Part model, mm, in its own coordinate system. A direction names the side the tool comes from. Round coordinates to 2 decimals unless told otherwise and drop trailing zeros. Write each loop counter-clockwise with the first axis right and the second up, starting at its lowest first coordinate (ties: lowest second). Pieces come first, ordered by that corner, then holes.
from build123d import *

# Parameters (mm, degrees)
SKETCH_2_R          = 2.1
CUT_EXTRUDE_1_DEPTH = 48.333920184
SKETCH_3_R          = 2.1
CUT_EXTRUDE_2_DEPTH = 53.389073288
EXTRUDE_1_DEPTH     = 4
FILLET_1_R          = 5


with BuildPart() as part:
    # 草图1 → 旋转1 (revolve)
    with BuildSketch(Plane(origin=(0, 0, 0), x_dir=(1, 0, 0), z_dir=(0, 1, 0)), mode=Mode.PRIVATE) as revolve_1_sk:
        Polygon((0, 21.25), (0, 23.75), (12, 23.75), (12, 31.5), (16, 31.5), (16, 23.75), (29.45, 23.75), (29.45, 13.01), (25.45, 13.01), (25.45, 21.25), align=None)
    revolve(revolve_1_sk.sketch.rotate(Axis((-873.269597079, 0, 0), (1, 0, 0)), 180), axis=Axis((-873.269597079, 0, 0), (1, 0, 0)))

    # 草图2 → 切除-拉伸1 (cut, through all)
    with BuildSketch(Plane(origin=(16, 0, 0), x_dir=(0, 0, -1), z_dir=(1, 0, 0))):
        with Locations((0, 27.75)):
            Circle(SKETCH_2_R)
        with Locations((-24.032204955, 13.875)):
            Circle(SKETCH_2_R)
        with Locations((-24.032204955, -13.875)):
            Circle(SKETCH_2_R)
        with Locations((0, -27.75)):
            Circle(SKETCH_2_R)
        with Locations((24.032204955, -13.875)):
            Circle(SKETCH_2_R)
        with Locations((24.032204955, 13.875)):
            Circle(SKETCH_2_R)
        with BuildLine():
            ThreePointArc((31.5, 0), (31.059418861, 5.25), (29.75, 10.35313962))
            Line((29.75, 10.35313962), (29.75, -10.35313962))
            ThreePointArc((29.75, -10.35313962), (31.059418861, -5.25), (31.5, 0))
        make_face()
        with BuildLine():
            ThreePointArc((23.84108192, 20.587685952), (15.75, 27.279800219), (5.90891808, 30.940825573))
            Line((5.90891808, 30.940825573), (23.84108192, 20.587685952))
        make_face()
        with BuildLine():
            Line((-23.84108192, 20.587685952), (-5.90891808, 30.940825573))
            ThreePointArc((-5.90891808, 30.940825573), (-15.75, 27.279800219), (-23.84108192, 20.587685952))
        make_face()
        with BuildLine():
            Line((-29.75, -10.35313962), (-29.75, 10.35313962))
            ThreePointArc((-29.75, 10.35313962), (-31.5, 0), (-29.75, -10.35313962))
        make_face()
        with BuildLine():
            Line((-5.90891808, -30.940825573), (-23.84108192, -20.587685952))
            ThreePointArc((-23.84108192, -20.587685952), (-15.75, -27.279800219), (-5.90891808, -30.940825573))
        make_face()
        with BuildLine():
            ThreePointArc((5.90891808, -30.940825573), (15.75, -27.279800219), (23.84108192, -20.587685952))
            Line((23.84108192, -20.587685952), (5.90891808, -30.940825573))
        make_face()
    extrude(amount=-CUT_EXTRUDE_1_DEPTH, mode=Mode.SUBTRACT)

    # 草图3 → 切除-拉伸2 (cut, through all)
    with BuildSketch(Plane(origin=(29.45, 0, 0), x_dir=(0, 0, -1), z_dir=(1, 0, 0))):
        with Locations((0, 17.5)):
            Circle(SKETCH_3_R)
        with Locations((17.5, 0)):
            Circle(SKETCH_3_R)
        with Locations((0, -17.5)):
            Circle(SKETCH_3_R)
        with Locations((-17.5, 0)):
            Circle(SKETCH_3_R)
    extrude(amount=-CUT_EXTRUDE_2_DEPTH, mode=Mode.SUBTRACT)

    # 草图2<3> → 凸台-拉伸1 (add)
    with BuildSketch(Plane(origin=(16, 0, 0), x_dir=(0, 0, -1), z_dir=(1, 0, 0))):
        with BuildLine():
            ThreePointArc((-29.75, 10.35313962), (-27.279800219, 15.75), (-23.84108192, 20.587685952))
            Line((-23.84108192, 20.587685952), (-29.75, 17.176170508))
            Line((-29.75, 17.176170508), (-29.75, 10.35313962))
        make_face()
        with BuildLine():
            Line((5.90891808, 30.940825573), (0, 34.352341017))
            Line((0, 34.352341017), (-5.90891808, 30.940825573))
            ThreePointArc((-5.90891808, 30.940825573), (0, 31.5), (5.90891808, 30.940825573))
        make_face()
        with BuildLine():
            Line((29.75, 17.176170508), (23.84108192, 20.587685952))
            ThreePointArc((23.84108192, 20.587685952), (27.279800219, 15.75), (29.75, 10.35313962))
            Line((29.75, 10.35313962), (29.75, 17.176170508))
        make_face()
        with BuildLine():
            Line((29.75, -17.176170508), (29.75, -10.35313962))
            ThreePointArc((29.75, -10.35313962), (27.279800219, -15.75), (23.84108192, -20.587685952))
            Line((23.84108192, -20.587685952), (29.75, -17.176170508))
        make_face()
        with BuildLine():
            ThreePointArc((5.90891808, -30.940825573), (0, -31.5), (-5.90891808, -30.940825573))
            Line((-5.90891808, -30.940825573), (0, -34.352341017))
            Line((0, -34.352341017), (5.90891808, -30.940825573))
        make_face()
        with BuildLine():
            ThreePointArc((-23.84108192, -20.587685952), (-27.279800219, -15.75), (-29.75, -10.35313962))
            Line((-29.75, -10.35313962), (-29.75, -17.176170508))
            Line((-29.75, -17.176170508), (-23.84108192, -20.587685952))
        make_face()
    extrude(amount=-EXTRUDE_1_DEPTH)

    # 圆角1
    fillet_1_edges = [part.edges().sort_by_distance(p)[0] for p in [
        (14, -17.176170508, 29.75),
        (14, -34.352341017, 0),
        (14, -17.176170508, -29.75),
        (14, 17.176170508, -29.75),
        (14, 34.352341017, 0),
        (14, 17.176170508, 29.75),
    ]]
    fillet(fillet_1_edges, radius=FILLET_1_R)


solid = part.part
Q1. Saw through at A-A, the plane y = 0. Write the cut outline in (x, z), and give its area (3 significant figures).
Q2. Two-plate mould, pull along Y, no slides. Class faces 4 (the cylindrical face through (14.03, 13.07, -25.97)), 5 (the cylindrical face through (13.972, -16.821, 29.062)), 6 (the flat face through (0, 12, 18)): released by +Y, released by -Y, zero draft, split by the parting line, or undercut.
Q3. Saw through at B-B, the plane y = 27.75. Write the cut outline in (x, z).
Q4. Tool access for faces 1 (the cylindrical face through (22.819, 23.185, -5.149)), 2 (the cylindrical face through (13.972, 16.821, -29.062)), 3 (the flat face through (12, 20.1, -13.1)): list every direction of +Z, -Z, +X, -X, +Y, -Y with a clear straight run to the whole face (end or side of a thin tool).
Q5. Saw through at C-C, the plane z = 0. Give the number of separate pieces and of enclosed holes in the cut face, and give its area (3 significant figures).
Q6. Wall check: line 1 (Y direction, x = 27.7, z = 0); line 2 (Y direction, x = 11.25, z = 0); line 3 (Y direction, x = 13.6, z = 0). Give the ranges that are in metal, low to high.
Q7. Drop flat-ended pins along their axis: P1, Ø4, axis at x = 21.5, z = -14, coming from the +Y side; P2, Ø3, axis at x = 21, z = 6, coming from the -Y side; P3, Ø10, axis at x = 24, z = 10, coming from the +Y side. Give the stop position or say it passes through.
Q8. Saw through at D-D, the plane z = 16.5. Write the cut outline in (x, y), and give its area (3 significant figures).
Computed:
1. outline: (0, -23.75) - (12, -23.75) - (12, -29.75) - (16, -29.75) - (16, -23.75) - (29.45, -23.75) - (29.45, -19.6) - (25.45, -19.6) - (25.45, -21.25) - (0, -21.25) - close; (0, 21.25) - (25.45, 21.25) - (25.45, 19.6) - (29.45, 19.6) - (29.45, 23.75) - (16, 23.75) - (16, 29.75) - (12, 29.75) - (12, 23.75) - (0, 23.75) - close; (25.45, -15.4) - (29.45, -15.4) - (29.45, -13.01) - (25.45, -13.01) - close; (25.45, 13.01) - (29.45, 13.01) - (29.45, 15.4) - (25.45, 15.4) - close
1. area: 228 mm2
2. face 4: undercut
2. face 5: released by -Y
2. face 6: zero draft
3. outline: (12, -11.44) - (16, -11.44) - (16, -2.1) - (12, -2.1) - close; (12, 2.1) - (16, 2.1) - (16, 11.44) - (12, 11.44) - close
4. face 1: +X
4. face 2: -Z, +X, -X, +Y
4. face 3: -X
5. separate pieces: 6
5. enclosed holes: 0
5. area: 225 mm2
6. line 1: y = -23.75 to -19.6, -15.4 to -13.01, 13.01 to 15.4, 19.6 to 23.75
6. line 2: y = -23.75 to -21.25, 21.25 to 23.75
6. line 3: y = -33.58 to -29.85, -25.65 to -21.25, 21.25 to 25.65, 29.85 to 33.58
7. P1: stops at y = 20.5
7. P2: stops at y = -23.32
7. P3: stops at y = 23.22
8. outline: (0, -17.08) - (12, -17.08) - (12, -24.83) - (16, -24.83) - (16, -17.08) - (29.45, -17.08) - (29.45, -1.85) - (25.45, -1.85) - (25.45, -13.39) - (0, -13.39) - close; (0, 13.39) - (25.45, 13.39) - (25.45, 1.85) - (29.45, 1.85) - (29.45, 17.08) - (16, 17.08) - (16, 24.83) - (12, 24.83) - (12, 17.08) - (0, 17.08) - close
8. area: 372 mm2
